Verification items for the finished model (mm, model axes). Face numbers are marked on the shaded views. A direction names the side the tool comes from. Coordinates: 2 decimals unless noted, no trailing zeros. Write each loop counter-clockwise with the first axis right and the second up, starting at its lowest first coordinate (ties: lowest second). Pieces come first, ordered by that corner, then holes. Notation, with made-up numbers: (84, -5.5) -> (120, -5.5) arc R18 ccw to (120, 9.5) -> close; hole circle Ø7 at (46.5, 51.25). An arc over 180 degrees is marked (long way). Answer in a Markdown table with one row per item.
```python
from build123d import *

# Parameters (mm, degrees)
BOSS_EXTRUDE2_DEPTH = 2.5
SKETCH5_W           = 63.43934648
SKETCH5_H           = 13.991199956
BOSS_EXTRUDE3_DEPTH = 30
FILLET1_R           = 5
SKETCH6_R           = 2
CUT_EXTRUDE1_DEPTH  = 162.963105911


with BuildPart() as part:
    # Sketch2 → Boss-Extrude2 (new, symmetric)
    with BuildSketch(Plane(origin=(0, 0, 0), x_dir=(1, 0, 0), z_dir=(0, 1, 0))):
        with BuildLine():
            Line((-50, 30), (50, 30))
            Line((50, 30), (150, 30))
            Line((150, 30), (150, 28))
            ThreePointArc((150, 28), (122, 0), (150, -28))
            Line((150, -28), (150, -30))
            Line((150, -30), (50, -30))
            Line((50, -30), (-50, -30))
            Line((-50, -30), (-50, 30))
        make_face()
    extrude(amount=BOSS_EXTRUDE2_DEPTH, both=True)

    # Sketch5 → Boss-Extrude3 (add, symmetric)
    with BuildSketch(Plane.XY):
        with Locations((-81.71967324, 4.495599978)):
            Rectangle(SKETCH5_W, SKETCH5_H)
    extrude(amount=BOSS_EXTRUDE3_DEPTH, both=True)

    # Fillet1
    fillet1_edges = [part.edges().sort_by_distance(p)[0] for p in [
        (-50, 2.5, 0),
    ]]
    fillet(fillet1_edges, radius=FILLET1_R)

    # Sketch6 → Cut-Extrude1 (cut, through all)
    with BuildSketch(Plane.XY.offset(30)):
        with Locations((-95.43934648, 5.491199956)):
            Circle(SKETCH6_R)
    extrude(amount=-CUT_EXTRUDE1_DEPTH, mode=Mode.SUBTRACT)


solid = part.part
```
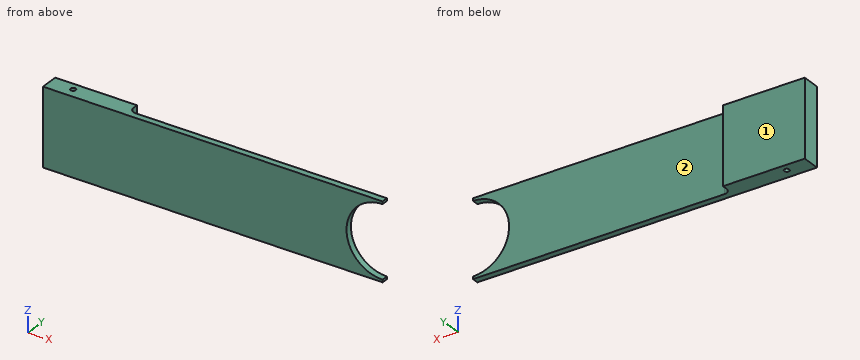
1. Tool access check on the marked faces 1 and 2. Record the directions out of +Z, -Z, +X, -X, +Y, -Y that give a thin tool (end or side, any length) a straight path to the whole face; none if there is none.
Geometry says:
| item | result |
|---|---|
| face 1 | +Z, -Z, +X, -X, +Y |
| face 2 | +Z, -Z, +X, +Y |
2. Depth check by flat-ended pin: P1, Ø5, axis at x = 110, z = 10.5, coming from the +Y side; P2, Ø2, axis at y = 10, z = 13.5, coming from the +X side; P3, Ø3, axis at y = 2.5, z = 16.5, coming from the +X side. Enter the tip coordinate at first touch or a pass-through.
Geometry says:
| item | result |
|---|---|
| P1 | y = 2.5 |
| P2 | x = -50 |
| P3 | x = 128.55 |
3. Section check B-B, the plane x = -19.5. Record the boundary of the cut face in (y, z), plus the area to 3 significant figures.
Geometry says:
| item | result |
|---|---|
| outline | (-2.5, -30) -> (2.5, -30) -> (2.5, 30) -> (-2.5, 30) -> close |
| area | 300 mm^2 |
4. Section check A-A, the plane z = 20. Record the boundary of the cut face in (x, y), plus the area to 3 significant figures.
Geometry says:
| item | result |
|---|---|
| outline | (-113.44, -2.5) -> (130.4, -2.5) -> (130.4, 2.5) -> (-45, 2.5) arc R5 cw to (-50, 7.5) -> (-50, 11.49) -> (-113.44, 11.49) -> close; hole circle Ø4 at (-95.44, 5.49) |
| area | 1,780 mm^2 |
5. Section check C-C, the plane z = -19. Record the boundary of the cut face in (x, y).
Geometry says:
| item | result |
|---|---|
| outline | (-113.44, -2.5) -> (129.43, -2.5) -> (129.43, 2.5) -> (-45, 2.5) arc R5 cw to (-50, 7.5) -> (-50, 11.49) -> (-113.44, 11.49) -> close; hole circle Ø4 at (-95.44, 5.49) |
6. Thickness scan on line 1 (Y direction, x = 32, z = -15.5); line 2 (X direction, y = 10.75, z = -3.5); line 3 (X direction, y = 6.5, z = -9). Record the ranges inside material, lowest first. Write a range as from..to.
Geometry says:
| item | result |
|---|---|
| line 1 | -2.5..2.5 |
| line 2 | -113.44..-50 |
| line 3 | -113.44..-97.17, -93.71..-49.9 |
